Part model, mm, in its own coordinate system. A direction names the side the tool comes from. Give positions to 0.01 mm unless a question says otherwise; leave off trailing zeros. Write each loop counter-clockwise with the first axis right and the second up, starting at its lowest first coordinate (ties: lowest second). Pieces come first, ordered by that corner, then holes. Notation, with made-up numbers: M 31.25,-20.5 L 71.25,-20.5 A30 cw 71.25,5.5 Z; hole C -5.75,15.5 d4. An arc over 180 degrees is marked long. Use a Markdown table: item, result. Add a question column.
from build123d import *

# Parameters (mm, degrees)
SKETCH1_W           = 35
SKETCH1_H           = 65
SKETCH1_R           = 13.75
BOSS_EXTRUDE1_DEPTH = 12
CHAMFER1_SIZE       = 10
SKETCH2_W           = 55
SKETCH2_H           = 10
BOSS_EXTRUDE2_DEPTH = 25
SKETCH3_W           = 35
SKETCH3_H           = 6
CUT_EXTRUDE1_DEPTH  = 52.188768299
CUT_EXTRUDE2_DEPTH  = 13.5
CHAMFER2_SIZE       = 0.5
SKETCH5_W           = 1
SKETCH5_H           = 37.783958766
CUT_EXTRUDE3_DEPTH  = 52.188768299
SKETCH6_R           = 5
CUT_EXTRUDE4_DEPTH  = 10
SKETCH7_R           = 2.25
CUT_EXTRUDE5_DEPTH  = 7
M4_TAPPED_HOLE1_D   = 3.3


with BuildPart() as part:
    # Sketch1 → Boss-Extrude1 (new body)
    with BuildSketch(Plane(origin=(0, 0, 0), x_dir=(1, 0, 0), z_dir=(0, 1, 0))):
        with Locations((0, -2.7)):
            Rectangle(SKETCH1_W, SKETCH1_H)
        with Locations(Location((0, 0, 0), (0, 0, 270))):
            Circle(SKETCH1_R, mode=Mode.SUBTRACT)
    extrude(amount=BOSS_EXTRUDE1_DEPTH)

    # Chamfer1
    chamfer1_edges = [part.edges().sort_by_distance(p)[0] for p in [
        (-17.5, 6, -29.8),
        (17.5, 6, -29.8),
    ]]
    chamfer(chamfer1_edges, length=CHAMFER1_SIZE)

    # Sketch2 → Boss-Extrude2 (add)
    with BuildSketch(Plane(origin=(0, 12, 0), x_dir=(1, 0, 0), z_dir=(0, 1, 0))):
        with Locations((0, -30.2)):
            Rectangle(SKETCH2_W, SKETCH2_H)
    extrude(amount=-BOSS_EXTRUDE2_DEPTH)

    # Sketch3 → Cut-Extrude1 (cut, through all)
    with BuildSketch(Plane.XZ.offset(13)):
        with Locations((0, 35.2)):
            Rectangle(SKETCH3_W, SKETCH3_H)
    extrude(amount=-CUT_EXTRUDE1_DEPTH, mode=Mode.SUBTRACT)

    # Sketch4 → Cut-Extrude2 (cut)
    with BuildSketch(Plane(origin=(0, 0, 25.2), x_dir=(-1, 0, 0), z_dir=(0, 0, -1))):
        with BuildLine():
            Line((-20.75, 8.5), (-20.75, 3.5))
            ThreePointArc((-20.75, 3.5), (-23, 1.25), (-25.25, 3.5))
            Line((-25.25, 3.5), (-25.25, 8.5))
            ThreePointArc((-25.25, 8.5), (-23, 10.75), (-20.75, 8.5))
        make_face()
        with BuildLine():
            Line((20.75, 8.5), (20.75, 3.5))
            ThreePointArc((20.75, 3.5), (23, 1.25), (25.25, 3.5))
            Line((25.25, 3.5), (25.25, 8.5))
            ThreePointArc((25.25, 8.5), (23, 10.75), (20.75, 8.5))
        make_face()
        with BuildLine():
            Line((20.75, -9.5), (20.75, -4.5))
            ThreePointArc((20.75, -4.5), (23, -2.25), (25.25, -4.5))
            Line((25.25, -4.5), (25.25, -9.5))
            ThreePointArc((25.25, -9.5), (23, -11.75), (20.75, -9.5))
        make_face()
        with BuildLine():
            Line((-20.75, -9.5), (-20.75, -4.5))
            ThreePointArc((-20.75, -4.5), (-23, -2.25), (-25.25, -4.5))
            Line((-25.25, -4.5), (-25.25, -9.5))
            ThreePointArc((-25.25, -9.5), (-23, -11.75), (-20.75, -9.5))
        make_face()
    extrude(amount=-CUT_EXTRUDE2_DEPTH, mode=Mode.SUBTRACT)

    # Chamfer2
    chamfer2_edges = [part.edges().sort_by_distance(p)[0] for p in [
        (17.5, -0.5, 35.2),
        (-17.5, -0.5, 35.2),
    ]]
    chamfer(chamfer2_edges, length=CHAMFER2_SIZE)

    # Sketch5 → Cut-Extrude3 (cut, through all)
    with BuildSketch(Plane(origin=(0, 12, 0), x_dir=(1, 0, 0), z_dir=(0, 1, 0))):
        with Locations((0, 29.8)):
            Rectangle(SKETCH5_W, SKETCH5_H)
    extrude(amount=-CUT_EXTRUDE3_DEPTH, mode=Mode.SUBTRACT)

    # Sketch6 → Cut-Extrude4 (cut)
    with BuildSketch(Plane.ZY.offset(17.5)):
        with Locations((-21.8, 6)):
            Circle(SKETCH6_R)
    extrude(amount=-CUT_EXTRUDE4_DEPTH, mode=Mode.SUBTRACT)

    # Sketch7 → Cut-Extrude5 (cut)
    with BuildSketch(Plane.ZY.offset(7.5)):
        with Locations((-21.8, 6)):
            Circle(SKETCH7_R)
    extrude(amount=-CUT_EXTRUDE5_DEPTH, mode=Mode.SUBTRACT)

    # M4 Tapped Hole1 (through all)
    with Locations(Plane.ZY.offset(-0.5)):
        with Locations((-21.8, 6)):
            Hole(M4_TAPPED_HOLE1_D / 2)


solid = part.part
1. Cut at D-D (z = -21.8). Write the cut outline in (x, y), then the cut area to 3 significant figures.
2. Mould opens along X. For faces 1 (the flat face through (-17.5, -1, 33)), 2 (the cylindrical face through (9.02, 6.07, -20.15)), 3 (the flat face through (-27.5, 0, 30)), 4 (the flat face through (0, -1, 32.2)) say: released by +X, released by -X, zero draft, split by the parting line, or undercut.
3. Cut at A-A (y = -6.5). Write the cut outline in (x, z).
4. Tool access for faces 5 (the flat face through (-0.5, 9, -22)), 6 (the flat face through (-17.5, 6, 3)), 7 (the flat face through (17.5, -1, 33)), 8 (the cylindrical face through (-22.95, -2.25, 30.13)): list every direction of +Z, -Z, +X, -X, +Y, -Y with a clear straight run to the whole face (end or side of a thin tool).
5. Flat gauge pins, fed straight in: pin 1 (6 mm diameter, centred on y = 6, z = -21.8, fed in from +X); pin 2 (3.5 mm diameter, centred on y = 7, z = -18, fed in from -X); pin 3 (3 mm diameter, centred on x = -6.5, z = -19, fed in from -Y). Where does each tip first touch, or does it go through?
6. Drill centre lines: probe 1 along Y at (x, z) = (-5.5, -21.8); probe 2 along Z at (x, y) = (4.5, 6); probe 3 along Y at (x, z) = (8.5, -21.8). Where is each one in solid material? Low to high. Write a range as [from, to].
7. Cut at C-C (x = 23). Write the cut outline in (y, z), then the cut area to 3 significant figures.
8. Cut at B-B (z = 0). Write the cut outline in (x, y), then the cut area to 3 significant figures.
A:
| question | item | result |
|---|---|---|
| 1 | outline | M -15.5,0 L -0.5,0 L -0.5,3.75 L -7.5,3.75 L -7.5,1 L -15.5,1 Z; M -15.5,11 L -7.5,11 L -7.5,8.25 L -0.5,8.25 L -0.5,12 L -15.5,12 Z; M 0.5,0 L 15.5,0 L 15.5,4.35 L 0.5,4.35 Z; M 0.5,7.65 L 15.5,7.65 L 15.5,12 L 0.5,12 Z |
| 1 | area | 199 mm² |
| 2 | face 1 | undercut |
| 2 | face 2 | zero draft |
| 2 | face 3 | released by -X |
| 2 | face 4 | undercut |
| 3 | outline | M -27.5,25.2 L -25.25,25.2 L -25.25,35.2 L -27.5,35.2 Z; M -20.75,25.2 L 20.75,25.2 L 20.75,35.2 L 18,35.2 L 17.5,34.7 L 17.5,32.2 L -17.5,32.2 L -17.5,34.7 L -18,35.2 L -20.75,35.2 Z; M 25.25,25.2 L 27.5,25.2 L 27.5,35.2 L 25.25,35.2 Z |
| 4 | face 5 | -Z, +Y, -Y |
| 4 | face 6 | -Z, -X, +Y, -Y |
| 4 | face 7 | +Z, +Y, -Y |
| 4 | face 8 | +Z, -Z |
| 5 | pin 1 | stops at x = 17.5 |
| 5 | pin 2 | stops at x = -17.5 |
| 5 | pin 3 | stops at y = 0 |
| 6 | probe 1 | y = [0, 3.75], [8.25, 12] |
| 6 | probe 2 | z = [-29.8, -23.45], [-20.15, -12.99], [12.99, 32.2] |
| 6 | probe 3 | y = [0, 4.35], [7.65, 12] |
| 7 | outline | M -13,25.2 L -11.75,25.2 L -11.75,35.2 L -13,35.2 Z; M -2.25,25.2 L 1.25,25.2 L 1.25,35.2 L -2.25,35.2 Z; M 10.75,25.2 L 12,25.2 L 12,35.2 L 10.75,35.2 Z |
| 7 | area | 60.0 mm² |
| 8 | outline | M -17.5,0 L -13.75,0 L -13.75,12 L -17.5,12 Z; M 13.75,0 L 17.5,0 L 17.5,12 L 13.75,12 Z |
| 8 | area | 90.0 mm² |
